from build123d import *

# Parameters (mm, degrees)
SKETCH1_W             = 42
SKETCH1_H             = 45
SKETCH1_R             = 6
SKETCH1_R_2           = 1.5
BOSS_EXTRUDE1_DEPTH   = 6
SKETCH3_R             = 8
CUT_EXTRUDE1_DEPTH    = 5
SKETCH4_R             = 1.5
CUT_EXTRUDE2_DEPTH    = 32.356817441
SKETCH5_R             = 2.5
CUT_EXTRUDE3_DEPTH    = 4
SKETCH6_R             = 1
CUT_EXTRUDE4_DEPTH    = 2
M3_TAPPED_HOLE1_D     = 2.5
M3_TAPPED_HOLE1_DEPTH = 7.5
M3_TAPPED_HOLE1_TIP   = 0.751075774


with BuildPart() as part:
    # Sketch1 → Boss-Extrude1 (new body)
    with BuildSketch(Plane(origin=(0, 0, 0), x_dir=(1, 0, 0), z_dir=(0, 1, 0))):
        Rectangle(SKETCH1_W, SKETCH1_H)
        with Locations(Location((0, 8.5, 0), (0, 0, 270))):
            Circle(SKETCH1_R, mode=Mode.SUBTRACT)
        with Locations(Location((0, -6.5, 0), (0, 0, 270))):
            Circle(SKETCH1_R_2, mode=Mode.SUBTRACT)
    extrude(amount=BOSS_EXTRUDE1_DEPTH)

    # Sketch3 → Cut-Extrude1 (cut)
    with BuildSketch(Plane(origin=(0, 6, 0), x_dir=(1, 0, 0), z_dir=(0, 1, 0))):
        with Locations(Location((0, 8.5, 0), (0, 0, 270))):
            Circle(SKETCH3_R)
    extrude(amount=-CUT_EXTRUDE1_DEPTH, mode=Mode.SUBTRACT)

    # Sketch4 → Cut-Extrude2 (cut, through all)
    with BuildSketch(Plane(origin=(0, 6, 0), x_dir=(1, 0, 0), z_dir=(0, 1, 0))):
        with Locations(Location((-17.5, -17.5, 0), (0, 0, 270))):
            Circle(SKETCH4_R)
        with Locations(Location((17.5, -17.5, 0), (0, 0, 270))):
            Circle(SKETCH4_R)
    extrude(amount=-CUT_EXTRUDE2_DEPTH, mode=Mode.SUBTRACT)

    # Sketch5 → Cut-Extrude3 (cut)
    with BuildSketch(Plane.XZ):
        with Locations(Location((17.5, 17.5, 0), (0, 0, 270))):
            Circle(SKETCH5_R)
        with Locations(Location((-17.5, 17.5, 0), (0, 0, 270))):
            Circle(SKETCH5_R)
    extrude(amount=-CUT_EXTRUDE3_DEPTH, mode=Mode.SUBTRACT)

    # Sketch6 → Cut-Extrude4 (cut)
    with BuildSketch(Plane(origin=(21, 0, 0), x_dir=(0, 0, -1), z_dir=(1, 0, 0))):
        with Locations((6.5, 3)):
            Circle(SKETCH6_R)
        with Locations((-3, 3)):
            Circle(SKETCH6_R)
    extrude(amount=-CUT_EXTRUDE4_DEPTH, mode=Mode.SUBTRACT)

    # M3 Tapped Hole1
    with Locations(Plane(origin=(21, 0, 0), x_dir=(0, 0, -1), z_dir=(1, 0, 0))):
        with Locations((6.5, 3), (-3, 3)):
            Hole(M3_TAPPED_HOLE1_D / 2, depth=M3_TAPPED_HOLE1_DEPTH)
            with Locations((0, 0, -(M3_TAPPED_HOLE1_DEPTH + M3_TAPPED_HOLE1_TIP / 2))):  # 118° drill point
                Cone(0, M3_TAPPED_HOLE1_D / 2, M3_TAPPED_HOLE1_TIP, mode=Mode.SUBTRACT)


solid = part.part
Verification items for the finished model (mm, model axes). A direction names the side the tool comes from. Round coordinates to 2 decimals unless told otherwise and drop trailing zeros. Order: outer loops, then holes, each group sorted by start corner. A loop starts at its lowest first (then second) coordinate and runs counter-clockwise, first axis right, second up. Notation, with made-up numbers: (71, -3.5) -> (121, -3.5) arc R27 cw to (121, 16.5) -> close; hole circle Ø8 at (64.5, -13). An arc over 180 degrees is marked (long way). Put each result on its own line as item: value.
1) Section check C-C (x = 0). Record the cut outline in (y, z).
Final values:
outline: (0, -22.5) -> (6, -22.5) -> (6, -16.5) -> (1, -16.5) -> (1, -14.5) -> (0, -14.5) -> close; (0, -2.5) -> (1, -2.5) -> (1, -0.5) -> (6, -0.5) -> (6, 5) -> (0, 5) -> close; (0, 8) -> (6, 8) -> (6, 22.5) -> (0, 22.5) -> close
2) Section check D-D (x = -17.5). Record the cut outline in (y, z), then the cut area to 3 significant figures.
Final values:
outline: (0, -22.5) -> (6, -22.5) -> (6, 16) -> (4, 16) -> (4, 15) -> (0, 15) -> close; (0, 20) -> (4, 20) -> (4, 19) -> (6, 19) -> (6, 22.5) -> (0, 22.5) -> close
area: 244 mm^2
3) Mould release check, pull along Y, two halves, no side actions. Record for faces 6 (the flat face through (6, 1, -7)), 7 (the conical face through (12.88, 3.01, 3.22)), 8 (the cylindrical face through (-17.4, 2, 20)): +Y half, -Y half, draft (parallel to the pull), parting line (faces both ways), or undercut.
Final values:
face 6: +Y half
face 7: undercut
face 8: draft
4) Section check B-B (z = 6.5). Record the cut outline in (x, y).
Final values:
outline: (-21, 0) -> (-1.5, 0) -> (-1.5, 6) -> (-21, 6) -> close; (1.5, 0) -> (21, 0) -> (21, 6) -> (1.5, 6) -> close
5) Set-up check for faces 1 (the flat face through (-19, 4, 16)), 2 (the cylindrical face through (-4.868, 3.535, -14.849)), 3 (the cylindrical face through (17.2, 3.05, -7.75)), 4 (the flat face through (0, 3, -22.5)), 5 (the cylindrical face through (1.802, 0.493, -2.777)): record each of +Z, -Z, +X, -X, +Y, -Y from which the full face is reachable in a straight line by a thin tool's end or side.
Final values:
face 1: -Y
face 2: +Y
face 3: +X
face 4: -Z, +X, -X, +Y, -Y
face 5: +Y, -Y
6) Depth check by flat-ended pin: pin 1 (2.5 mm diameter, centred on x = -16.5, z = 17, fed in from -Y); pin 2 (11 mm diameter, centred on x = 0, z = -8.5, fed in from -Y). Enter the tip coordinate at first touch or a pass-through.
Final values:
pin 1: stops at y = 4
pin 2: passes through
7) Material ranges on line 1 (Y direction, x = 18, z = 3); line 2 (X direction, y = 1.7, z = 6.5); line 3 (X direction, y = 0.65, z = -8.5), recorded low to high.
Final values:
line 1: y = 0 to 1.75, 4.25 to 6
line 2: x = -21 to -1.5, 1.5 to 21
line 3: x = -21 to -6, 6 to 21
8) Section check A-A (x = 17.5). Record the cut outline in (y, z), then the cut area to 3 significant figures.
Final values:
outline: (0, -22.5) -> (6, -22.5) -> (6, 16) -> (4, 16) -> (4, 15) -> (0, 15) -> close; (0, 20) -> (4, 20) -> (4, 19) -> (6, 19) -> (6, 22.5) -> (0, 22.5) -> close; hole circle Ø2.5 at (3, -6.5); hole circle Ø2.5 at (3, 3)
area: 234 mm^2
